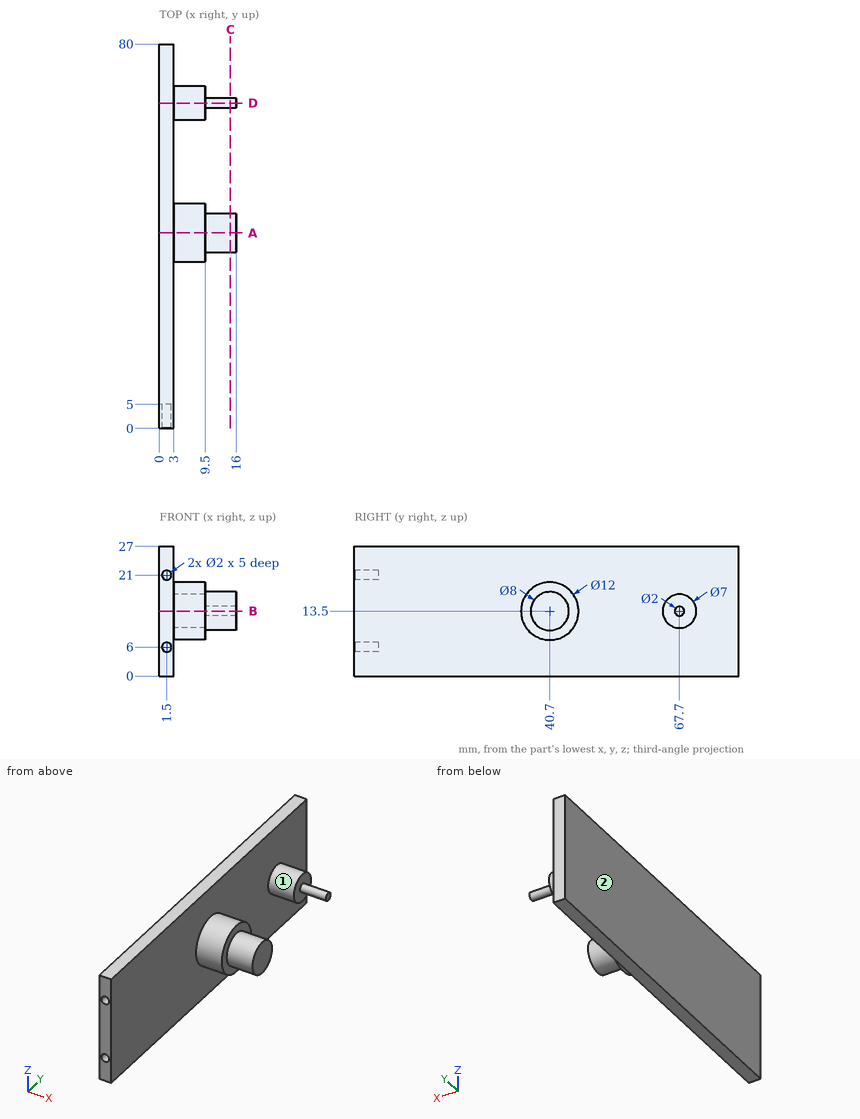
For this review, use the dimensioned drawing (mm, ordinates from the lowest corner) and the shaded views. A direction names the side the tool comes from. Give positions to 0.01 mm unless a question says otherwise; leave off trailing zeros. Loops run counter-clockwise (first coordinate to the right, second up) from the corner with the lowest first, then second, coordinate; pieces in that order, holes last. Notation, with made-up numbers: (-27, -4) - (-20, -4) arc R13 ccw to (-20, 20) - close; hole circle Ø5 at (52.5, -30.75). An arc over 180 degrees is marked (long way). Write each question's results on one line, items separated by ' | '.
(1) For the marked faces 1 and 2, list the 3-axis set-ups (+Z, -Z, +X, -X, +Y, -Y) from which the entire face can be reached by the end or side of a thin tool; tool diameter is ignored.
Conclusion:
face 1: +X | face 2: +Z, -Z, -X, +Y, -Y
(2) Take a section at C-C (x = 14.75). Give the boundary of the cut face in (y, z), then the cut area to 3 significant figures.
Conclusion:
outline: circle Ø8 at (40.7, 13.5); circle Ø2 at (67.7, 13.5) | area: 53.4 mm^2
(3) Take a section at D-D (y = 67.7). Give the boundary of the cut face in (x, z), then the cut area to 4 significant figures.
Conclusion:
outline: (0, 0) - (3, 0) - (3, 10) - (9.5, 10) - (9.5, 12.5) - (16, 12.5) - (16, 14.5) - (9.5, 14.5) - (9.5, 17) - (3, 17) - (3, 27) - (0, 27) - close | area: 139.5 mm^2
(4) Take a section at A-A (y = 40.7). Give the boundary of the cut face in (x, z), then the cut area to 3 significant figures.
Conclusion:
outline: (0, 0) - (3, 0) - (3, 7.5) - (9.5, 7.5) - (9.5, 9.5) - (16, 9.5) - (16, 17.5) - (9.5, 17.5) - (9.5, 19.5) - (3, 19.5) - (3, 27) - (0, 27) - close | area: 211 mm^2
(5) Take a section at B-B (z = 13.5). Give the boundary of the cut face in (x, y).
Conclusion:
outline: (0, 0) - (3, 0) - (3, 34.7) - (9.5, 34.7) - (9.5, 36.7) - (16, 36.7) - (16, 44.7) - (9.5, 44.7) - (9.5, 46.7) - (3, 46.7) - (3, 64.2) - (9.5, 64.2) - (9.5, 66.7) - (16, 66.7) - (16, 68.7) - (9.5, 68.7) - (9.5, 71.2) - (3, 71.2) - (3, 80) - (0, 80) - close
(6) For line 1 along Z through (x, y) = (1.5, 1); line 2 along X through (y, z) = (54, 17.75); line 3 along Y through (x, z) = (13.25, 13.75), list the stretches that pass through material, from the lowest coordinate up.
Conclusion:
line 1: 0 to 5, 7 to 20, 22 to 27 | line 2: 0 to 3 | line 3: 36.71 to 44.69, 66.73 to 68.67
(7) For pin 1 Ø1.5 at (x, z) = (8, 18.5) entering from -Y; pin 2 Ø1 at (y, z) = (46, 14.5) entering from +X; pin 3 Ø0.6 at (x, z) = (1.5, 20.5) entering from -Y, all flat-tipped, find the tip position at first contact; note any pin that passes through.
Conclusion:
pin 1: y = 36.46 | pin 2: x = 9.5 | pin 3: y = 5
